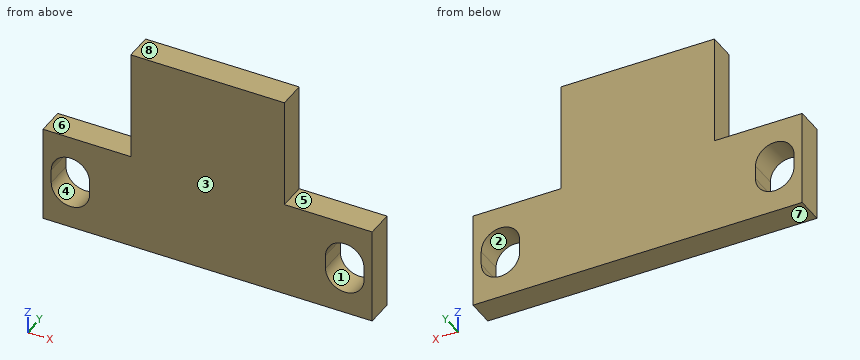
```python
from build123d import *

# Parameters (mm, degrees)
BOSS_EXTRUDE1_DEPTH = 10


with BuildPart() as part:
    # Sketch1 → Boss-Extrude1 (new body)
    with BuildSketch(Plane(origin=(0, 0, 0), x_dir=(1, 0, 0), z_dir=(0, 1, 0))):
        Polygon((-60, 37.5), (-60, 2.5), (-28, 2.5), (-28, -37.5), (28, -37.5), (28, 2.5), (60, 2.5), (60, 37.5), align=None)
        with BuildLine():
            ThreePointArc((-57, 22.5), (-50, 29.5), (-43, 22.5))
            Line((-43, 22.5), (-43, 17.5))
            ThreePointArc((-43, 17.5), (-50, 10.5), (-57, 17.5))
            Line((-57, 17.5), (-57, 22.5))
        make_face(mode=Mode.SUBTRACT)
        with BuildLine():
            Line((43, 17.5), (43, 22.5))
            ThreePointArc((43, 22.5), (50, 29.5), (57, 22.5))
            Line((57, 22.5), (57, 17.5))
            ThreePointArc((57, 17.5), (50, 10.5), (43, 17.5))
        make_face(mode=Mode.SUBTRACT)
    extrude(amount=BOSS_EXTRUDE1_DEPTH)


solid = part.part
```
Verification items for the finished model (mm, model axes). Face numbers are marked on the shaded views. A direction names the side the tool comes from. Coordinates: 2 decimals unless noted, no trailing zeros. Loops run counter-clockwise (first coordinate to the right, second up) from the corner with the lowest first, then second, coordinate; pieces in that order, holes last. Notation, with made-up numbers: (-13.75, 57) -> (36.25, 57) arc R19 cw to (36.25, 79) -> close; hole circle Ø7 at (59.5, -17). An arc over 180 degrees is marked (long way). Answer in a Markdown table with one row per item. Add a question column.
1. Access from +Z, -Z, +X, -X, +Y, -Y to the whole of each face (thin tool, end or side, straight path). Record for the marked faces 4, 5, 6, 7 and 8.
2. Depth check by flat-ended pin: P1, Ø5, axis at y = 6.5, z = 11, coming from the -X side; P2, Ø3, axis at y = 3.5, z = 14.5, coming from the +X side; P3, Ø3, axis at x = -44, y = 5, coming from the +Z side. Enter the tip coordinate at first touch or a pass-through.
3. Material ranges on probe 1 along Z at (x, y) = (-36, 6); probe 2 along X at (y, z) = (6, 3); probe 3 along X at (y, z) = (0.5, -13), recorded low to high. Write a range as [from, to].
4. Section check B-B, the plane z = -15. Enter the section's corners in (x, y).
5. Section check A-A, the plane x = 50. Enter the section's corners in (y, z), then the cut area to 3 significant figures.
6. Draft check along X on the marked faces 1, 2 and 3. Enter one of: +X half, -X half, draft (parallel to the pull), parting line (faces both ways), or undercut.
7. Section check D-D, the plane z = 16.5. Enter the section's corners in (x, y), then the cut area to 3 significant figures.
8. Section check C-C, the plane y = 4. Enter the section's corners in (x, z), then the cut area to 3 significant figures.
Derived:
| question | item | result |
|---|---|---|
| 1 | face 4 | +Y, -Y |
| 1 | face 5 | +Z, +X, +Y, -Y |
| 1 | face 6 | +Z, -X, +Y, -Y |
| 1 | face 7 | -Z, +X, -X, +Y, -Y |
| 1 | face 8 | +Z, +X, -X, +Y, -Y |
| 2 | P1 | stops at x = -28 |
| 2 | P2 | stops at x = 28 |
| 2 | P3 | stops at z = -2.5 |
| 3 | probe 1 | z = [-37.5, -2.5] |
| 3 | probe 2 | x = [-28, 28] |
| 3 | probe 3 | x = [-60, -55.36], [-44.64, 44.64], [55.36, 60] |
| 4 | outline | (-60, 0) -> (-56.54, 0) -> (-56.54, 10) -> (-60, 10) -> close; (-43.46, 0) -> (43.46, 0) -> (43.46, 10) -> (-43.46, 10) -> close; (56.54, 0) -> (60, 0) -> (60, 10) -> (56.54, 10) -> close |
| 5 | outline | (0, -37.5) -> (10, -37.5) -> (10, -29.5) -> (0, -29.5) -> close; (0, -10.5) -> (10, -10.5) -> (10, -2.5) -> (0, -2.5) -> close |
| 5 | area | 160 mm² |
| 6 | face 1 | undercut |
| 6 | face 2 | undercut |
| 6 | face 3 | draft |
| 7 | outline | (-28, 0) -> (28, 0) -> (28, 10) -> (-28, 10) -> close |
| 7 | area | 560 mm² |
| 8 | outline | (-60, -37.5) -> (60, -37.5) -> (60, -2.5) -> (28, -2.5) -> (28, 37.5) -> (-28, 37.5) -> (-28, -2.5) -> (-60, -2.5) -> close; hole (-57, -22.5) arc R7 ccw to (-43, -22.5) -> (-43, -17.5) arc R7 ccw to (-57, -17.5) -> close; hole (43, -22.5) arc R7 ccw to (57, -22.5) -> (57, -17.5) arc R7 ccw to (43, -17.5) -> close |
| 8 | area | 5,990 mm² |
